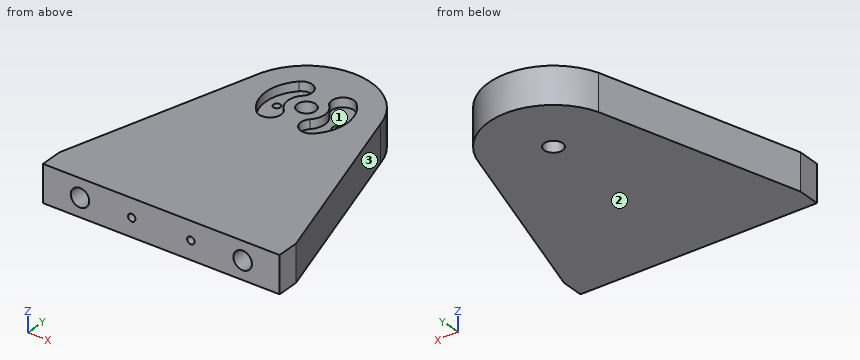
```python
from build123d import *

# Parameters (mm, degrees)
POST_PLATE_10MM_DEPTH       = 10
UPPER_SLOT_PROFILE_R        = 2.5
UPPER_SLOT_CUT_DEPTH        = 10
UPPER_SLOT_RELIEF_PROFILE_R = 2.1
UPPER_SLOT_RELIEF_CUT_DEPTH = 12.4
LONG_SLOT_PROFILE_R         = 1
LONG_SLOT_CUT_55_DEEP_DEPTH = 55
SHAFT_BORE_5_PROFILE_R      = 2.5
SHAFT_BORE_5_DEPTH          = 55
PIVOT_RECESS_2_5_DEEP_DEPTH = 2.5
LOWER_SLOT_PROFILE_R        = 1
LOWER_SLOT_CUT_DEPTH        = 5


with BuildPart() as part:
    # Post Plate Profile → Post Plate 10mm (new body)
    with BuildSketch(Plane.XY):
        with BuildLine():
            Line((-32, 0), (32, 0))
            Line((32, 0), (32, 6))
            Line((32, 6), (17.027168619, 57.040486211))
            ThreePointArc((17.027168619, 57.040486211), (0.915873878, 70.476017139), (-16.511549747, 58.798165653))
            Line((-16.511549747, 58.798165653), (-32, 6))
            Line((-32, 6), (-32, 0))
        make_face()
    extrude(amount=POST_PLATE_10MM_DEPTH)

    # Upper Slot Profile → Upper Slot Cut (cut)
    with BuildSketch(Plane.XZ):
        with Locations(Location((22, 5, 0), (0, 0, 270))):
            Circle(UPPER_SLOT_PROFILE_R)
        with Locations(Location((-22, 5, 0), (0, 0, 270))):
            Circle(UPPER_SLOT_PROFILE_R)
    extrude(amount=-UPPER_SLOT_CUT_DEPTH, mode=Mode.SUBTRACT)

    # Upper Slot Relief Profile → Upper Slot Relief Cut (cut)
    with BuildSketch(Plane.XZ):
        with Locations(Location((22, 5, 0), (0, 0, 270))):
            Circle(UPPER_SLOT_RELIEF_PROFILE_R)
        with Locations(Location((-22, 5, 0), (0, 0, 270))):
            Circle(UPPER_SLOT_RELIEF_PROFILE_R)
    extrude(amount=-UPPER_SLOT_RELIEF_CUT_DEPTH, mode=Mode.SUBTRACT)

    # Long Slot Profile → Long Slot Cut 55 Deep (cut)
    with BuildSketch(Plane.XZ):
        with Locations(Location((-8, 5, 0), (0, 0, 270))):
            Circle(LONG_SLOT_PROFILE_R)
        with Locations(Location((8, 5, 0), (0, 0, 270))):
            Circle(LONG_SLOT_PROFILE_R)
    extrude(amount=-LONG_SLOT_CUT_55_DEEP_DEPTH, mode=Mode.SUBTRACT)

    # Shaft Bore Ø5 Profile → Shaft Bore Ø5 (cut)
    with BuildSketch(Plane.XY.offset(10)):
        with Locations((0, 53)):
            Circle(SHAFT_BORE_5_PROFILE_R)
    extrude(amount=-SHAFT_BORE_5_DEPTH, mode=Mode.SUBTRACT)

    # Pivot Recess Profile → Pivot Recess 2.5 Deep (cut)
    with BuildSketch(Plane.XY.offset(10)):
        with BuildLine():
            ThreePointArc((-3.535533906, 56.535533906), (-5, 53), (-3.535533906, 49.464466094))
            ThreePointArc((-3.535533906, 49.464466094), (-3.535533906, 45.221825407), (-7.778174593, 45.221825407))
            ThreePointArc((-7.778174593, 45.221825407), (-11, 53), (-7.778174593, 60.778174593))
            ThreePointArc((-7.778174593, 60.778174593), (-3.535533906, 60.778174593), (-3.535533906, 56.535533906))
        make_face()
        with BuildLine():
            ThreePointArc((7.778174593, 45.221825407), (11, 53), (7.778174593, 60.778174593))
            ThreePointArc((7.778174593, 60.778174593), (3.535533906, 60.778174593), (3.535533906, 56.535533906))
            ThreePointArc((3.535533906, 56.535533906), (5, 53), (3.535533906, 49.464466094))
            ThreePointArc((3.535533906, 49.464466094), (3.535533906, 45.221825407), (7.778174593, 45.221825407))
        make_face()
    extrude(amount=-PIVOT_RECESS_2_5_DEEP_DEPTH, mode=Mode.SUBTRACT)

    # Lower Slot Profile → Lower Slot Cut (cut)
    with BuildSketch(Plane.XY.offset(7.5)):
        with Locations((8, 53)):
            Circle(LOWER_SLOT_PROFILE_R)
        with Locations((-8, 53)):
            Circle(LOWER_SLOT_PROFILE_R)
    extrude(amount=-LOWER_SLOT_CUT_DEPTH, mode=Mode.SUBTRACT)


solid = part.part
```
The model under review builds one solid part; all positions refer to its coordinate system, in mm. Face numbers are marked on the shaded views. Round coordinates to 2 decimals unless told otherwise and drop trailing zeros. Write each loop counter-clockwise with the first axis right and the second up, starting at its lowest first coordinate (ties: lowest second). Pieces come first, ordered by that corner, then holes. Notation, with made-up numbers: (36, 45) -> (73, 45) arc R12 cw to (73, 54) -> close; hole circle Ø9 at (66, 36.5). An arc over 180 degrees is marked (long way). Use CSV: the item, a comma, the result in double quotes.
Q1. Consider section C-C (x = 21). Give the boundary of the cut face in (y, z), then the cut area to 3 significant figures.
Checks:
outline,"(0, 0) -> (43.5, 0) -> (43.5, 10) -> (0, 10) -> (0, 7.29) -> (10, 7.29) -> (10, 6.85) -> (12.4, 6.85) -> (12.4, 3.15) -> (10, 3.15) -> (10, 2.71) -> (0, 2.71) -> close"
area,"380 mm²"
Q2. To check wall thickness, follow probe 1 along X at (y, z) = (2.75, 5); probe 2 along X at (y, z) = (11.2, 5); probe 3 along X at (y, z) = (53.6, 5). State the ranges of each line that lie inside material, in increasing order. Write a range as [from, to].
Checks:
probe 1,"[-32, -24.5], [-19.5, -9], [-7, 7], [9, 19.5], [24.5, 32]"
probe 2,"[-30.47, -24.1], [-19.9, -9], [-7, 7], [9, 19.9], [24.1, 30.47]"
probe 3,"[-18.04, -9], [-7, -2.43], [2.43, 7], [9, 18.04]"
Q3. Consider section B-B (y = 43.5). Give the boundary of the cut face in (x, z).
Checks:
outline,"(-21, 0) -> (21, 0) -> (21, 10) -> (-21, 10) -> close; hole circle Ø2 at (-8, 5); hole circle Ø2 at (8, 5)"
Q4. Mouldability with a two-part tool opening along Y and no side actions: class the marked faces 1, 2 and 3 as released by +Y, released by -Y, zero draft, split by the parting line, or undercut.
Checks:
face 1,"undercut"
face 2,"zero draft"
face 3,"released by +Y"
Q5. For pin 1 Ø3 at (x, y) = (8, 53) entering from +Z; pin 2 Ø5 at (y, z) = (15, 4) entering from +X; pin 3 Ø1.6 at (x, z) = (-8, 5) entering from -Y, all flat-tipped, find the tip position at first contact; note any pin that passes through.
Checks:
pin 1,"z = 7.5"
pin 2,"x = 30.09"
pin 3,"y = 55"
Q6. Consider section A-A (x = 0). Give the boundary of the cut face in (y, z).
Checks:
outline,"(0, 0) -> (50.5, 0) -> (50.5, 10) -> (0, 10) -> close; (55.5, 0) -> (70.5, 0) -> (70.5, 10) -> (55.5, 10) -> close"
Q7. Consider section D-D (y = 31). Give the boundary of the cut face in (x, z).
Checks:
outline,"(-24.67, 0) -> (24.67, 0) -> (24.67, 10) -> (-24.67, 10) -> close; hole circle Ø2 at (-8, 5); hole circle Ø2 at (8, 5)"
